Geometry check sheet. Reference: the model listing, model coordinates, mm. A direction names the side the tool comes from. Round coordinates to 2 decimals unless told otherwise and drop trailing zeros. Order: outer loops, then holes, each group sorted by start corner. A loop starts at its lowest first (then second) coordinate and runs counter-clockwise, first axis right, second up. Notation, with made-up numbers: (-13, -28.75) - (16, -28.75) arc R31 ccw to (16, 1.25) - close; hole circle Ø7 at (21, -23). An arc over 180 degrees is marked (long way). Use a Markdown table: item, result. Add a question column.
(1) Section check B-B on z = 38. Record the boundary of the cut face in (x, y), then the cut area to 3 significant figures.
(2) Access from +Z, -Z, +X, -X, +Y, -Y to the whole of each face (thin tool, end or side, straight path). Record for faces 1 (the face through (75, 47, 50)), 2 (the face through (50, 25, 12)), 3 (the face through (75, 25, 75)).
(3) Mould release check, pull along Z, two halves, no side actions. Record for faces 4 (the face through (75, 25, 28)), 5 (the face through (75, 25, 25)), 6 (the face through (50, 25, 87)): released by +Z, released by -Z, zero draft, split by the parting line, or undercut.
(4) Gauge pin test, flat ends, axial feed: P1, Ø25, axis at x = 82.5, y = 13, coming from the -Z side; P2, Ø12, axis at y = 7, z = 15.5, coming from the +X side; P3, Ø25, axis at x = 87, y = 17.5, coming from the +Z side. Record the tip position at first contact, or that the pin passes through.
(5) Section check D-D on x = 28.5. Record the boundary of the cut face in (y, z).
(6) Section check A-A on y = 42. Record the boundary of the cut face in (x, z).
(7) Thickness scan on line 1 along Y through (x, z) = (93, 70.5); line 2 along Z through (x, y) = (63.5, 33). Record the ranges inside material, lowest first. Write a range as [from, to].
(8) Section check C-C on x = 59. Record the boundary of the cut face in (y, z).
```python
from build123d import *

# Parameters (mm, degrees)
SKETCH_1_W          = 50
SKETCH_1_H          = 50
SKETCH_1_W_2        = 44
SKETCH_1_H_2        = 44
EXTRUDE_1_DEPTH     = 200
SKETCH_2_W          = 56
SKETCH_2_H          = 56
CUT_EXTRUDE_1_DEPTH = 100
EXTRUDE_3_DEPTH     = 100
SKETCH_4_W          = 44
SKETCH_4_H          = 44
CUT_EXTRUDE_2_DEPTH = 100


with BuildPart() as part:
    # 草图1 → 凸台-拉伸1 (new body)
    with BuildSketch(Plane.XY):
        with Locations((25, 25)):
            Rectangle(SKETCH_1_W, SKETCH_1_H)
        with Locations((25, 25)):
            Rectangle(SKETCH_1_W_2, SKETCH_1_H_2, mode=Mode.SUBTRACT)
    extrude(amount=EXTRUDE_1_DEPTH)

    # 草图2 → 切除-拉伸1 (cut)
    with BuildSketch(Plane.XY.offset(200)):
        with Locations((25, 25)):
            Rectangle(SKETCH_2_W, SKETCH_2_H)
    extrude(amount=-CUT_EXTRUDE_1_DEPTH, mode=Mode.SUBTRACT)

    # 草图3 → 凸台-拉伸3 (add)
    with BuildSketch(Plane.ZY):
        Polygon((50, 50), (25, 50), (25, 0), (75, 0), (75, 50), align=None)
        Polygon((50, 47), (28, 47), (28, 3), (72, 3), (72, 47), align=None, mode=Mode.SUBTRACT)
    extrude(amount=-EXTRUDE_3_DEPTH)

    # 草图4 → 切除-拉伸2 (cut)
    with BuildSketch(Plane(origin=(0, 0, 0), x_dir=(-1, 0, 0), z_dir=(0, 0, -1))):
        with Locations((-25, 25)):
            Rectangle(SKETCH_4_W, SKETCH_4_H)
    extrude(amount=-CUT_EXTRUDE_2_DEPTH, mode=Mode.SUBTRACT)


solid = part.part
```
Check sheet entries:
| question | item | result |
|---|---|---|
| 1 | outline | (0, 0) - (100, 0) - (100, 3) - (50, 3) - (50, 47) - (100, 47) - (100, 50) - (0, 50) - close; hole (3, 3) - (47, 3) - (47, 47) - (3, 47) - close |
| 1 | area | 864 mm2 |
| 2 | face 1 | +X |
| 2 | face 2 | -Z, +X, +Y, -Y |
| 2 | face 3 | +Z, +X, +Y, -Y |
| 3 | face 4 | undercut |
| 3 | face 5 | released by -Z |
| 3 | face 6 | zero draft |
| 4 | P1 | stops at z = 25 |
| 4 | P2 | stops at x = 50 |
| 4 | P3 | stops at z = 75 |
| 5 | outline | (0, 0) - (3, 0) - (3, 100) - (0, 100) - close; (47, 0) - (50, 0) - (50, 100) - (47, 100) - close |
| 6 | outline | (0, 0) - (3, 0) - (3, 100) - (0, 100) - close; (47, 0) - (50, 0) - (50, 25) - (100, 25) - (100, 28) - (50, 28) - (50, 72) - (100, 72) - (100, 75) - (50, 75) - (50, 100) - (47, 100) - close |
| 7 | line 1 | y = [0, 3], [47, 50] |
| 7 | line 2 | z = [25, 28], [72, 75] |
| 8 | outline | (0, 25) - (50, 25) - (50, 75) - (0, 75) - close; hole (3, 28) - (47, 28) - (47, 72) - (3, 72) - close |
